Work out the finished part from the listing and answer in its coordinate system (mm). Round coordinates to 2 decimals unless told otherwise and drop trailing zeros. Loops run counter-clockwise (first coordinate to the right, second up) from the corner with the lowest first, then second, coordinate; pieces in that order, holes last. Notation, with made-up numbers: (21.5, 44) - (34.5, 44) arc R14 ccw to (34.5, 65) - close; hole circle Ø5 at (24.25, 17). An arc over 180 degrees is marked (long way). Answer as CSV lines item,"result". Start each with the question number.
Q1. Section C-C on x = 6 is taken. Write down the section's boundary in (y, z).
Q2. Straight lines are drawn through the part: L1, parallel to Y at x = -6, z = 1.95; L2, parallel to X at y = -6.5, z = 2.15; L3, parallel to X at y = 20.5, z = 1.2. For each, find the intervals that lie inside material, in ascending order. Write a range as [from, to].
Q3. The mould has two halves that part along X. Classify faces 1 (the face through (-26, 0, 3)), 2 (the face through (-8.15, 0.09, 1.52)), 3 (the face through (-79, -20, 2)): +X half, -X half, draft (parallel to the pull), parting line (faces both ways), or undercut.
Q4. Section A-A on y = -8 is taken. Write down the section's boundary in (x, z).
Q5. Section D-D on z = 1.25 is taken. Write down the section's boundary in (x, y).
Q6. Section B-B on y = 12 is taken. Write down the section's boundary in (x, z), then the cut area to 3 significant figures.
```python
from build123d import *

# Parameters (mm, degrees)
SKETCH_1_W          = 160
SKETCH_1_H          = 44
EXTRUDE_1_DEPTH     = 3
SKETCH_2_R          = 7
SKETCH_2_R_2        = 2.15
CUT_EXTRUDE_1_DEPTH = 3
FILLET_1_R          = 5
SKETCH_3_W          = 63.678392254
SKETCH_3_H          = 72.512670224
CUT_EXTRUDE_2_DEPTH = 10
FILLET_2_R          = 5


with BuildPart() as part:
    # 草图1 → 凸台-拉伸1 (new body)
    with BuildSketch(Plane.XY):
        Rectangle(SKETCH_1_W, SKETCH_1_H)
    extrude(amount=EXTRUDE_1_DEPTH)

    # 草图2 → 切除-拉伸1 (cut)
    with BuildSketch(Plane.XY.offset(3)):
        with Locations((-62.5, -8)):
            Circle(SKETCH_2_R)
        with Locations((62.5, -8)):
            Circle(SKETCH_2_R)
        with Locations((-6, 12)):
            Circle(SKETCH_2_R_2)
        with Locations((6, 12)):
            Circle(SKETCH_2_R_2)
        with Locations((6, 0)):
            Circle(SKETCH_2_R_2)
        with Locations((-6, 0)):
            Circle(SKETCH_2_R_2)
    extrude(amount=-CUT_EXTRUDE_1_DEPTH, mode=Mode.SUBTRACT)

    # 圆角1
    fillet_1_edges = [part.edges().sort_by_distance(p)[0] for p in [
        (80, -22, 1.5),
        (-80, -22, 1.5),
        (-80, 22, 1.5),
        (80, 22, 1.5),
    ]]
    fillet(fillet_1_edges, radius=FILLET_1_R)

    # 草图3 → 切除-拉伸2 (cut)
    with BuildSketch(Plane.XY.offset(3)):
        with Locations((61.839196127, 0.092590352)):
            Rectangle(SKETCH_3_W, SKETCH_3_H)
    extrude(amount=-CUT_EXTRUDE_2_DEPTH, mode=Mode.SUBTRACT)

    # 圆角2
    fillet_2_edges = [part.edges().sort_by_distance(p)[0] for p in [
        (30, 22, 1.5),
        (30, -22, 1.5),
    ]]
    fillet(fillet_2_edges, radius=FILLET_2_R)


solid = part.part
```
Findings:
1,outline,"(-22, 0) - (-2.15, 0) - (-2.15, 3) - (-22, 3) - close; (2.15, 0) - (9.85, 0) - (9.85, 3) - (2.15, 3) - close; (14.15, 0) - (22, 0) - (22, 3) - (14.15, 3) - close"
2,L1,"y = [-22, -2.15], [2.15, 9.85], [14.15, 22]"
2,L2,"x = [-80, -69.34], [-55.66, 30]"
2,L3,"x = [-78.57, 28.57]"
3,face 1,"draft"
3,face 2,"undercut"
3,face 3,"-X half"
4,outline,"(-80, 0) - (-69.5, 0) - (-69.5, 3) - (-80, 3) - close; (-55.5, 0) - (30, 0) - (30, 3) - (-55.5, 3) - close"
5,outline,"(-80, -17) arc R5 ccw to (-75, -22) - (25, -22) arc R5 ccw to (30, -17) - (30, 17) arc R5 ccw to (25, 22) - (-75, 22) arc R5 ccw to (-80, 17) - close; hole circle Ø14 at (-62.5, -8); hole circle Ø4.3 at (-6, 0); hole circle Ø4.3 at (-6, 12); hole circle Ø4.3 at (6, 0); hole circle Ø4.3 at (6, 12)"
6,outline,"(-80, 0) - (-8.15, 0) - (-8.15, 3) - (-80, 3) - close; (-3.85, 0) - (3.85, 0) - (3.85, 3) - (-3.85, 3) - close; (8.15, 0) - (30, 0) - (30, 3) - (8.15, 3) - close"
6,area,"304 mm^2"
